Geometry: final body of the model. Coordinates: model frame, mm. Face numbers are marked on the shaded views. A direction names the side the tool comes from. Coordinates: 2 decimals unless noted, no trailing zeros. Loops run counter-clockwise (first coordinate to the right, second up) from the corner with the lowest first, then second, coordinate; pieces in that order, holes last. Notation, with made-up numbers: (51, 74) - (94, 74) arc R15 ccw to (94, 93) - close; hole circle Ø11 at (-3, -0.5). An arc over 180 degrees is marked (long way). Return JSON: item names as keys, results as strings.
from build123d import *

# Parameters (mm, degrees)
EXTRUDE_1_DEPTH     = 100
SKETCH_2_W          = 35.317953013
SKETCH_2_H          = 4.2
CUT_EXTRUDE_1_DEPTH = 60
RIB_6_REACH         = 112.526
SKETCH_5_WALL_W     = 269.149287264
SKETCH_5_WALL_H     = 10
SKETCH_6_R          = 3
CUT_EXTRUDE_2_DEPTH = 10
SKETCH_7_R          = 1
CUT_EXTRUDE_3_DEPTH = 15


with BuildPart() as part:
    # 草图1 → 凸台-拉伸1 (new body)
    with BuildSketch(Plane.XY):
        Polygon((-37.5, 32.788461538), (42.5, 32.788461538), (42.5, 22.788461538), (-27.5, 22.788461538), (-27.5, -37.211538462), (-37.5, -37.211538462), align=None)
    extrude(amount=EXTRUDE_1_DEPTH)

    # 草图2 → 切除-拉伸1 (cut)
    with BuildSketch(Plane.XY.offset(100)):
        with Locations((-12.799064643, 30.688461538)):
            Rectangle(SKETCH_2_W, SKETCH_2_H)
    extrude(amount=-CUT_EXTRUDE_1_DEPTH, mode=Mode.SUBTRACT)

    # 草图5 wall → 筋6 (add, up to next)
    with BuildSketch(Plane(origin=(-10, 7.788461538, 95), x_dir=(-0.759256602365, -0.650791373456, 0), z_dir=(0.650791373456, -0.759256602365, 0)), mode=Mode.PRIVATE) as rib_6_sk1:
        Rectangle(SKETCH_5_WALL_W, SKETCH_5_WALL_H)
    rib_6_tool1 = extrude(rib_6_sk1.sketch, amount=-RIB_6_REACH, mode=Mode.PRIVATE) - part.part
    add(rib_6_tool1.solids().sort_by_distance((-10, 7.788461538, 95))[0])

    # 草图6 → 切除-拉伸2 (cut)
    with BuildSketch(Plane(origin=(-27.5, 891.532711259, -866.3577183), x_dir=(0, 0, 1), z_dir=(1, 0, 0))):
        with Locations(Location((900.249826396, 880.97002325, 0), (0, 0, 270))):
            Circle(SKETCH_6_R)
        with Locations(Location((890.712774703, 880.97002325, 0), (0, 0, 270))):
            Circle(SKETCH_6_R)
        with Locations(Location((900.249826396, 913.137579673, 0), (0, 0, 270))):
            Circle(SKETCH_6_R)
        with Locations(Location((890.712774703, 913.137579673, 0), (0, 0, 270))):
            Circle(SKETCH_6_R)
    extrude(amount=-CUT_EXTRUDE_2_DEPTH, mode=Mode.SUBTRACT)

    # 草图7 → 切除-拉伸3 (cut)
    with BuildSketch(Plane(origin=(1081.455900364, 22.788461538, -866.3577183), x_dir=(-0.07845909572783148, 0, 0.9969173337331291), z_dir=(0, -1, 0))):
        with Locations(Location((963.085867609, 999.8129825, 0), (0, 0, 265.5))):
            Circle(SKETCH_7_R)
        with Locations(Location((977.974059883, 997.984942349, 0), (0, 0, 265.5))):
            Circle(SKETCH_7_R)
        with Locations(Location((961.501566145, 986.909882529, 0), (0, 0, 265.5))):
            Circle(SKETCH_7_R)
        with Locations(Location((976.389758419, 985.081842378, 0), (0, 0, 265.5))):
            Circle(SKETCH_7_R)
    extrude(amount=-CUT_EXTRUDE_3_DEPTH, mode=Mode.SUBTRACT)


solid = part.part
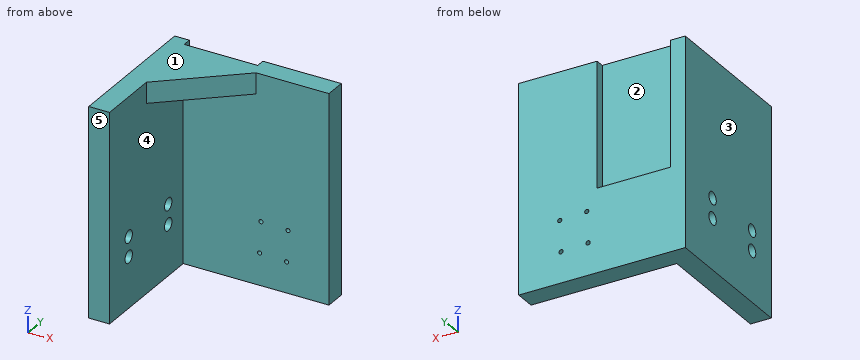
Item 1: Section query A-A, the plane z = 79. Return loops of the section in (x, y), and give its area (3 significant figures).
Worked out:
{"outline": "(-37.5, -37.21) - (-27.5, -37.21) - (-27.5, 22.79) - (42.5, 22.79) - (42.5, 32.79) - (4.86, 32.79) - (4.86, 28.59) - (-30.46, 28.59) - (-30.46, 32.79) - (-37.5, 32.79) - close", "area": "1,250 mm^2"}
Item 2: First-contact query: pin 1 Ø5 at (y, z) = (4, 43.5) entering from +X; pin 2 Ø9 at (x, y) = (-14, 10.5) entering from -Z; pin 3 Ø5.5 at (y, z) = (-21.6, 24.36) entering from -X; pin 4 Ø4.5 at (x, y) = (-6, 31) entering from +Z. Flat tips, straight axial feed; report the tip coordinate or a pass-through.
Worked out:
{"pin 1": "x = -27.5", "pin 2": "z = 90", "pin 3": "through", "pin 4": "z = 40"}
Item 3: Section query D-D, the plane y = -1.5. Return loops of the section in (x, z), and give its area (3 significant figures).
Worked out:
{"outline": "(-37.5, 0) - (-27.5, 0) - (-27.5, 90) - (-20.84, 90) - (-20.84, 100) - (-37.5, 100) - close", "area": "1,070 mm^2"}
Item 4: Ray query, probe 1 along Y at (x, z) = (27, 79); probe 2 along X at (y, z) = (-4, 9.5); probe 3 along X at (y, z) = (27.5, 14). Return the intervals inside material, ascending. Write a range as from..to.
Worked out:
{"probe 1": "22.79..32.79", "probe 2": "-37.5..-27.5", "probe 3": "-37.5..21.49, 22.81..42.5"}
Item 5: Section query C-C, the plane y = -14. Return loops of the section in (x, z).
Worked out:
{"outline": "(-37.5, 0) - (-27.5, 0) - (-27.5, 100) - (-37.5, 100) - close"}
Item 6: Mould query, pull axis X, two halves, no side actions, for the marked faces 1, 2 and 3. Classes: +X half, -X half, draft (parallel to the pull), parting line (faces both ways), or undercut.
Worked out:
{"face 1": "draft", "face 2": "undercut", "face 3": "-X half"}
Item 7: Section query B-B, the plane x = -17. Return loops of the section in (y, z).
Worked out:
{"outline": "(1.79, 90) - (22.79, 90) - (22.79, 0) - (32.79, 0) - (32.79, 40) - (28.59, 40) - (28.59, 100) - (1.79, 100) - close"}
Item 8: Reachability of the marked faces 4 and 5 from +Z, -Z, +X, -X, +Y, -Y: full face, straight path, thin tool, end or side. Return the list, or none.
Worked out:
{"face 4": "-Z, +X, -Y", "face 5": "+Z, -Z, +X, -X, -Y"}
